from build123d import *

# Parameters (mm, degrees)
BUSH_PROFILE_SKETCH_R   = 32.5
BUSH_BODY_DEPTH         = 40
FLANGE_PROFILE_SKETCH_R = 32.5
END_FLANGE_DEPTH        = 12.5


with BuildPart() as part:
    # Bush Profile Sketch → Bush Body (new, symmetric)
    with BuildSketch(Plane.XY):
        with BuildLine():
            Line((0, 40), (-44, 40))
            Line((-44, 40), (-44, -40))
            Line((-44, -40), (0, -40))
            ThreePointArc((0, -40), (40, 0), (0, 40))
        make_face()
        Circle(BUSH_PROFILE_SKETCH_R, mode=Mode.SUBTRACT)
    extrude(amount=BUSH_BODY_DEPTH, both=True)

    # Flange Profile Sketch → End Flange (add)
    with BuildSketch(Plane.XY.offset(40)):
        with BuildLine():
            Line((0, 48), (-52, 48))
            Line((-52, 48), (-52, -48))
            Line((-52, -48), (0, -48))
            ThreePointArc((0, -48), (48, 0), (0, 48))
        make_face()
        Circle(FLANGE_PROFILE_SKETCH_R, mode=Mode.SUBTRACT)
    end_flange = extrude(amount=END_FLANGE_DEPTH)

    # End Flange Mirror: End Flange across plane
    add(end_flange.mirror(Plane.XY))


solid = part.part
The listing builds one solid part. Answer for the finished solid, in the listing's coordinates (mm). A direction names the side the tool comes from. Give positions to 0.01 mm unless a question says otherwise; leave off trailing zeros. Loops run counter-clockwise (first coordinate to the right, second up) from the corner with the lowest first, then second, coordinate; pieces in that order, holes last. Notation, with made-up numbers: (48.5, 62.25) - (85.5, 62.25) arc R31 cw to (85.5, 88.25) - close; hole circle Ø10 at (-30.75, 8). An arc over 180 degrees is marked (long way). Write each question's results on one line, items separated by ' | '.
1. Find section D-D, the plane x = -37.5. Write down the section's boundary in (y, z), then the cut area to 3 significant figures.
Resolved:
outline: (-48, -52.5) - (48, -52.5) - (48, -40) - (40, -40) - (40, 40) - (48, 40) - (48, 52.5) - (-48, 52.5) - (-48, 40) - (-40, 40) - (-40, -40) - (-48, -40) - close | area: 8,800 mm^2
2. For a pull along Z with two mould halves and no side action, classify faces 1 (the face through (-26, -48, 46)), 2 (the face through (-22, -40, 1)), 3 (the face through (-25, 22, 52.5)) as +Z half, -Z half, draft (parallel to the pull), parting line (faces both ways), or undercut.
Resolved:
face 1: draft | face 2: undercut | face 3: +Z half
3. Consider probe 1 along Z at (x, y) = (41, 2); probe 2 along Y at (x, z) = (-6.5, -26.5); probe 3 along X at (y, z) = (19, -7). Determine where each line is inside the solid, lowest interval first. Write a range as from..to.
Resolved:
probe 1: z = -52.5..-40, 40..52.5 | probe 2: y = -40..-31.84, 31.84..40 | probe 3: x = -44..-26.37, 26.37..35.2
4. Find section A-A, the plane y = 0. Write down the section's boundary in (x, z), then the cut area to 4 significant figures.
Resolved:
outline: (-52, -52.5) - (-32.5, -52.5) - (-32.5, 52.5) - (-52, 52.5) - (-52, 40) - (-44, 40) - (-44, -40) - (-52, -40) - close; (32.5, -52.5) - (48, -52.5) - (48, -40) - (40, -40) - (40, 40) - (48, 40) - (48, 52.5) - (32.5, 52.5) - close | area: 2,395 mm^2
5. Flat-ended cylindrical pins translate along their axes: P1, Ø8, axis at x = -20, z = 24.5, coming from the +Y side; P2, Ø4, axis at x = 37.5, z = 27.5, coming from the +Y side; P3, Ø10, axis at y = -36.5, z = -33.5, coming from the -X side. Find the tip coordinate at first contact, or state that the pin passes through.
Resolved:
P1: stops at y = 40 | P2: stops at y = 18.43 | P3: stops at x = -44
6. Find section C-C, the plane x = 17. Write down the section's boundary in (y, z).
Resolved:
outline: (-44.89, -52.5) - (-27.7, -52.5) - (-27.7, 52.5) - (-44.89, 52.5) - (-44.89, 40) - (-36.21, 40) - (-36.21, -40) - (-44.89, -40) - close; (27.7, -52.5) - (44.89, -52.5) - (44.89, -40) - (36.21, -40) - (36.21, 40) - (44.89, 40) - (44.89, 52.5) - (27.7, 52.5) - close
7. Which of the six approach directions +Z, -Z, +X, -X, +Y, -Y give full straight-line access (tool end or side, diameter ignored) to faces 4 (the face through (-47, 4, 40)), 5 (the face through (-44, 1, 1)), 6 (the face through (-22, 40, 1))?
Resolved:
face 4: none | face 5: -X, +Y, -Y | face 6: +X, -X, +Y
8. Find section B-B, the plane z = -26. Write down the section's boundary in (x, y).
Resolved:
outline: (-44, -40) - (0, -40) arc R40 ccw to (0, 40) - (-44, 40) - close; hole circle Ø65 at (0, 0)
